Work out the finished part from the listing and answer in its coordinate system (mm). Coordinates: 2 decimals unless noted, no trailing zeros. Order: outer loops, then holes, each group sorted by start corner. A loop starts at its lowest first (then second) coordinate and runs counter-clockwise, first axis right, second up. Notation, with made-up numbers: M 31,-13 L 47,-13 A21 ccw 47,22 Z; hole C -7.5,30.25 d10. An arc over 180 degrees is marked long. Answer in a Markdown table with one row per item. Add a question column.
Item 1: The part is cut by section A-A (x = 0). Write down the section's boundary in (y, z), then the cut area to 3 significant figures.
Item 2: Consider line 1 (Y direction, x = 0, z = 0.5); line 2 (X direction, y = 1.5, z = 0.75); line 3 (X direction, y = 5, z = 0.1). Determine where each line is inside the solid, lowest interval first. Write a range as from..to.
Item 3: The part is cut by section C-C (x = -10.5). Write down the section's boundary in (y, z), then the cut area to 3 significant figures.
Item 4: The part is cut by section D-D (y = 20). Write down the section's boundary in (x, z).
Item 5: A flat-ended cylindrical pin translates along its axis: pin 1 Ø6 at (x, y) = (0, 20) entering from -Z. Find the tip coordinate at first contact, or state that the pin passes through.
from build123d import *

# Parameters (mm, degrees)
SKETCH1_R           = 27.5
SKETCH1_R_2         = 15
SKETCH1_R_3         = 3.25
BOSS_EXTRUDE1_DEPTH = 1


with BuildPart() as part:
    # Sketch1 → Boss-Extrude1 (new body)
    with BuildSketch(Plane.XY):
        Circle(SKETCH1_R)
        Circle(SKETCH1_R_2, mode=Mode.SUBTRACT)
        with Locations((0, 20)):
            Circle(SKETCH1_R_3, mode=Mode.SUBTRACT)
        with Locations((20, 0)):
            Circle(SKETCH1_R_3, mode=Mode.SUBTRACT)
        with Locations((0, -20)):
            Circle(SKETCH1_R_3, mode=Mode.SUBTRACT)
        with Locations((-20, 0)):
            Circle(SKETCH1_R_3, mode=Mode.SUBTRACT)
    extrude(amount=BOSS_EXTRUDE1_DEPTH)


solid = part.part
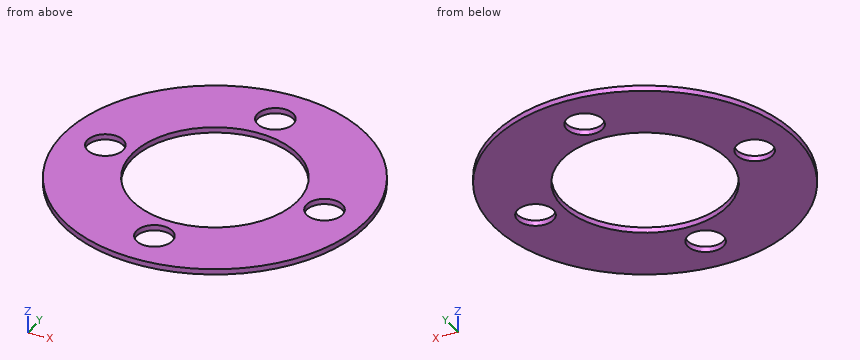
Reply:
| question | item | result |
|---|---|---|
| 1 | outline | M -27.5,0 L -23.25,0 L -23.25,1 L -27.5,1 Z; M -16.75,0 L -15,0 L -15,1 L -16.75,1 Z; M 15,0 L 16.75,0 L 16.75,1 L 15,1 Z; M 23.25,0 L 27.5,0 L 27.5,1 L 23.25,1 Z |
| 1 | area | 12.0 mm2 |
| 2 | line 1 | y = -27.5..-23.25, -16.75..-15, 15..16.75, 23.25..27.5 |
| 2 | line 2 | x = -27.46..-22.88, -17.12..-14.92, 14.92..17.12, 22.88..27.46 |
| 2 | line 3 | x = -27.04..-14.14, 14.14..27.04 |
| 3 | outline | M -25.42,0 L -10.71,0 L -10.71,1 L -25.42,1 Z; M 10.71,0 L 25.42,0 L 25.42,1 L 10.71,1 Z |
| 3 | area | 29.4 mm2 |
| 4 | outline | M -18.87,0 L -3.25,0 L -3.25,1 L -18.87,1 Z; M 3.25,0 L 18.87,0 L 18.87,1 L 3.25,1 Z |
| 5 | pin 1 | passes through |
